Model file for the job. Use its own axes, mm. Face numbers are marked on the shaded views. A direction names the side the tool comes from. Give positions to 0.01 mm unless a question says otherwise; leave off trailing zeros. Order: outer loops, then holes, each group sorted by start corner. A loop starts at its lowest first (then second) coordinate and runs counter-clockwise, first axis right, second up. Notation, with made-up numbers: M 27.25,-33 L 40.25,-33 A12 ccw 40.25,-25 Z; hole C 18.5,22 d10. An arc over 180 degrees is marked long. Return JSON: item names as keys, results as strings. Group by question number.
1. Slice it at C-C on y = 0. List the corners of the cut face in (x, z), then the cut area to 3 significant figures.
2. Wall check: probe 1 along X at (y, z) = (3, 6.75); probe 2 along Y at (x, z) = (0, 3); probe 3 along X at (y, z) = (19, 10.75). Give the ranges that are in metal, low to high. Write a range as [from, to].
3. Slice it at A-A on z = 10. List the corners of the cut face in (x, y).
4. Slice it at B-B on x = 0. List the corners of the cut face in (y, z), then the cut area to 3 significant figures.
5. Slice it at D-D on z = 26.25. List the corners of the cut face in (x, y).
6. Pin check, flat tips, straight feed: pin 1 (7.5 mm diameter, centred on x = -21.5, z = 8, fed in from +Y); pin 2 (8 mm diameter, centred on x = -18.5, y = -9, fed in from -Z); pin 3 (5.5 mm diameter, centred on x = -20, z = 10, fed in from -Y); pin 4 (23.5 mm diameter, centred on x = 0, y = 0, fed in from -Z). Stop position of each tip, or through.
7. 3-axis set-ups, long thin cutter, end or side, ignore diameter. For the marked faces 4, 5 and 6: which of +Z, -Z, +X, -X, +Y, -Y reach the whole face in a straight line?
8. Two-plate mould, pull along Z, no slides. Class the marked faces 1, 2 and 3: released by +Z, released by -Z, zero draft, split by the parting line, or undercut.
from build123d import *

# Parameters (mm, degrees)
SKETCH1_W                                            = 60
SKETCH1_H                                            = 45
SKETCH1_R                                            = 9
BOSS_EXTRUDE1_DEPTH                                  = 30
HOLE_SIZE_PER_SOCKET_HEAD_CAP_SCREW_TYPE_D           = 9
HOLE_SIZE_PER_SOCKET_HEAD_CAP_SCREW_TYPE_CBORE_D     = 15
HOLE_SIZE_PER_SOCKET_HEAD_CAP_SCREW_TYPE_CBORE_DEPTH = 9
SKETCH2_R                                            = 13.1
EXTRUDE1_DEPTH                                       = 9
EXTRUDE2_START                                       = -9
SKETCH3_R                                            = 13.1
EXTRUDE2_DEPTH                                       = 9


with BuildPart() as part:
    # Sketch1 → Boss-Extrude1 (new body)
    with BuildSketch(Plane.XY):
        with Locations((0, 2.5)):
            Rectangle(SKETCH1_W, SKETCH1_H)
        Circle(SKETCH1_R, mode=Mode.SUBTRACT)
    extrude(amount=BOSS_EXTRUDE1_DEPTH)

    # Hole size per socket head cap screw type1 (through all)
    with Locations(Plane(origin=(0, 25, 0), x_dir=(-1, 0, 0), z_dir=(0, 1, 0))):
        with Locations((20, 10), (-20, 10)):
            CounterBoreHole(HOLE_SIZE_PER_SOCKET_HEAD_CAP_SCREW_TYPE_D / 2, HOLE_SIZE_PER_SOCKET_HEAD_CAP_SCREW_TYPE_CBORE_D / 2, HOLE_SIZE_PER_SOCKET_HEAD_CAP_SCREW_TYPE_CBORE_DEPTH)

    # Sketch2 → Extrude1 (cut)
    with BuildSketch(Plane.XY.offset(30)):
        Circle(SKETCH2_R)
    extrude(amount=-EXTRUDE1_DEPTH, mode=Mode.SUBTRACT)

    # Sketch3 → Extrude2 (cut)
    with BuildSketch(Plane(origin=(0, 0, 0), x_dir=(-1, 0, 0), z_dir=(0, 0, -1)).offset(EXTRUDE2_START)):
        with Locations(Location((0, 0, 0), (0, 0, 180))):
            Circle(SKETCH3_R)
    extrude(amount=EXTRUDE2_DEPTH, mode=Mode.SUBTRACT)


solid = part.part
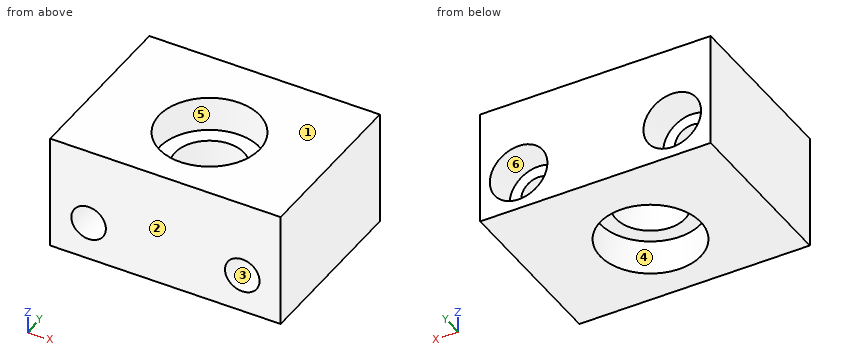
Result:
{
 "1": {"outline": "M -30,0 L -13.1,0 L -13.1,9 L -9,9 L -9,21 L -13.1,21 L -13.1,30 L -30,30 Z; M 9,9 L 13.1,9 L 13.1,0 L 30,0 L 30,30 L 13.1,30 L 13.1,21 L 9,21 Z; hole C -20,10 d9; hole C 20,10 d9", "area": "985 mm2"},
 "2": {"probe 1": "x = [-30, -23.11], [-16.89, -12.75], [12.75, 16.89], [23.11, 30]", "probe 2": "y = [-20, -13.1], [13.1, 25]", "probe 3": "x = [-30, -27.46], [-12.54, 12.54], [27.46, 30]"},
 "3": {"outline": "M -30,-20 L -24.5,-20 L -24.5,16 L -27.5,16 L -27.5,25 L -30,25 Z; M -15.5,-20 L 15.5,-20 L 15.5,16 L 12.5,16 L 12.5,25 L -12.5,25 L -12.5,16 L -15.5,16 Z; M 24.5,-20 L 30,-20 L 30,25 L 27.5,25 L 27.5,16 L 24.5,16 Z; hole C 0,0 d18"},
 "4": {"outline": "M -20,0 L -13.1,0 L -13.1,9 L -9,9 L -9,21 L -13.1,21 L -13.1,30 L -20,30 Z; M 9,9 L 13.1,9 L 13.1,0 L 25,0 L 25,30 L 13.1,30 L 13.1,21 L 9,21 Z", "area": "662 mm2"},
 "5": {"outline": "M -30,-20 L 30,-20 L 30,25 L -30,25 Z; hole C 0,0 d26.2"},
 "6": {"pin 1": "stops at y = 16", "pin 2": "stops at z = 0", "pin 3": "passes through", "pin 4": "stops at z = 9"},
 "7": {"face 4": "-Z", "face 5": "+Z", "face 6": "+Y"},
 "8": {"face 1": "released by +Z", "face 2": "zero draft", "face 3": "undercut"}
}
